Study the drawing (mm; zero at the part's minimum x, y, z) and answer. A direction names the side the tool comes from. Coordinates: 2 decimals unless noted, no trailing zeros. Write each loop counter-clockwise with the first axis right and the second up, starting at its lowest first coordinate (ties: lowest second). Pieces come first, ordered by that corner, then holes. Notation, with made-up numbers: M 4,33.5 L 28,33.5 A22 cw 28,54.5 Z; hole C 76,25.25 d11. An arc over 180 degrees is marked long. Answer as a JSON object with one key per item and string values. Group by question number.
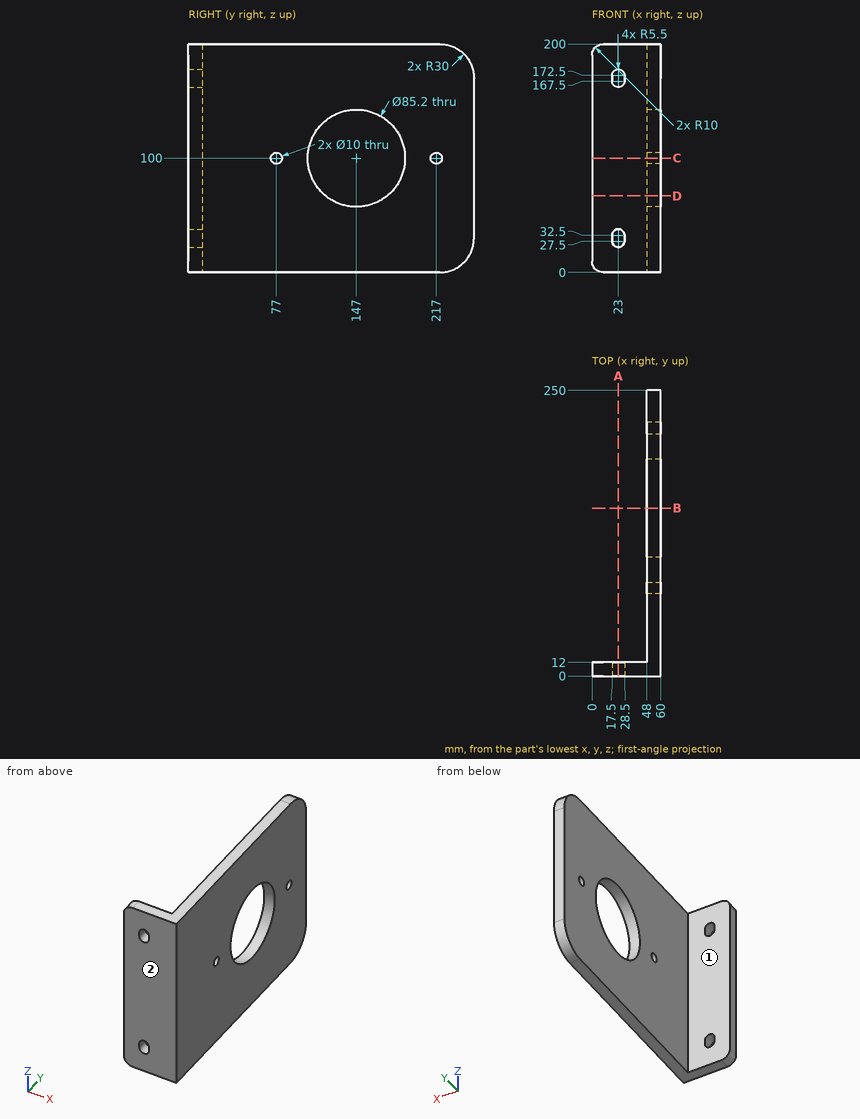
Item 1: A cutting plane is placed at A-A, the plane x = 23. Write down the section's boundary in (y, z).
Item 2: A cutting plane is placed at C-C, the plane z = 100. Write down the section's boundary in (x, y), and give its area (3 significant figures).
Item 3: A cutting plane is placed at D-D, the plane z = 67. Write down the section's boundary in (x, y).
Item 4: A tool of negligible diameter and unlimited length cuts with its end or side. For the marked faces 1 and 2, from which of +Z, -Z, +X, -X, +Y, -Y can it reach the whole face along a straight path? Write none if from no direction.
Item 5: Flat-ended cylindrical pins translate along their axes: pin 1 Ø1 at (y, z) = (25.5, 149) entering from -X; pin 2 Ø14.5 at (x, z) = (14, 58) entering from +Y. Find the tip coordinate at first contact, or state that the pin passes through.
Item 6: Consider L1, parallel to Z at x = 55, y = 217; L2, parallel to Y at x = 16, z = 67; L3, parallel to X at y = 124, z = 38. Determine where each line is inside the solid, lowest interval first. Write a range as from..to.
Item 7: A cutting plane is placed at B-B, the plane y = 147. Write down the section's boundary in (x, z).
Answer:
{
 "1": {"outline": "M 0,0 L 12,0 L 12,22 L 0,22 Z; M 0,38 L 12,38 L 12,162 L 0,162 Z; M 0,178 L 12,178 L 12,200 L 0,200 Z"},
 "2": {"outline": "M 0,0 L 60,0 L 60,72 L 48,72 L 48,12 L 0,12 Z; M 48,82 L 60,82 L 60,104.4 L 48,104.4 Z; M 48,189.6 L 60,189.6 L 60,212 L 48,212 Z; M 48,222 L 60,222 L 60,250 L 48,250 Z", "area": "2,310 mm2"},
 "3": {"outline": "M 0,0 L 60,0 L 60,120.06 L 48,120.06 L 48,12 L 0,12 Z; M 48,173.94 L 60,173.94 L 60,250 L 48,250 Z"},
 "4": {"face 1": "+Z, -Z, -X, +Y", "face 2": "+Z, -Z, +X, -X, -Y"},
 "5": {"pin 1": "x = 48", "pin 2": "y = 12"},
 "6": {"L1": "0..95, 105..200", "L2": "0..12", "L3": "48..60"},
 "7": {"outline": "M 48,0 L 60,0 L 60,57.4 L 48,57.4 Z; M 48,142.6 L 60,142.6 L 60,200 L 48,200 Z"}
}
